Work out the finished part from the listing and answer in its coordinate system (mm). A direction names the side the tool comes from. Coordinates: 2 decimals unless noted, no trailing zeros. Loops run counter-clockwise (first coordinate to the right, second up) from the corner with the lowest first, then second, coordinate; pieces in that order, holes last. Notation, with made-up numbers: (-21, 0) -> (25, 0) arc R36 cw to (25, 39) -> close; hole circle Ø8 at (38.5, 82.5). An arc over 180 degrees is marked (long way). Use a Markdown table: item, result.
from build123d import *

# Parameters (mm, degrees)
SKETCH_1_R               = 2.5
EXTRUDE_1_DEPTH          = 25
CHAMFER_1_SIZE           = 0.5
CUT_EXTRUDE_1_DEPTH      = 26.248762346
CUT_EXTRUDE_1_DEPTH_BACK = 26.248762346
SKETCH_2_W               = 3.2
SKETCH_2_H               = 3.525136196


with BuildPart() as part:
    # 草图1 → 凸台-拉伸1 (new, symmetric)
    with BuildSketch(Plane.XY):
        Circle(SKETCH_1_R)
    extrude(amount=EXTRUDE_1_DEPTH, both=True)

    # 倒角1
    chamfer_1_edges = [part.edges().sort_by_distance(p)[0] for p in [
        (-2.5, 0, -25),
        (-2.5, 0, 25),
    ]]
    chamfer(chamfer_1_edges, length=CHAMFER_1_SIZE)

    # 草图2 → 切除-拉伸1 (cut, two sides: drawn at the far end of the back side and taken through both)
    with BuildSketch(Plane(origin=(0, 0, 0), x_dir=(0, 0, -1), z_dir=(1, 0, 0)).offset(-CUT_EXTRUDE_1_DEPTH_BACK)):
        with Locations((21.4, 3.262568098)):
            Rectangle(SKETCH_2_W, SKETCH_2_H)
    extrude(amount=CUT_EXTRUDE_1_DEPTH + CUT_EXTRUDE_1_DEPTH_BACK, mode=Mode.SUBTRACT)


solid = part.part
Q1. Given pin 1 Ø2 at (x, z) = (1.5, -9.5) entering from +Y, flat-ended and moving along its own axis, determine where the tip first touches the part or whether it passes through.
Solved:
| item | result |
|---|---|
| pin 1 | y = 2.45 |
Q2. Consider line 1 (Z direction, x = -0.2, y = 1.55); line 2 (Y direction, x = -1.4, z = -17.5); line 3 (X direction, y = 1.75, z = 1). Determine where each line is inside the solid, lowest interval first. Write a range as [from, to].
Solved:
| item | result |
|---|---|
| line 1 | [-25, -23], [-19.8, 25] |
| line 2 | [-2.07, 2.07] |
| line 3 | [-1.79, 1.79] |
Q3. Section A-A on z = 16 is taken. Determine the outline of the cut face in (x, y), and give its area (3 significant figures).
Solved:
| item | result |
|---|---|
| outline | circle Ø5 at (0, 0) |
| area | 19.6 mm² |
Q4. For faces 1 (the cylindrical face through (1.15, -2.22, 0.34)), 2 (the flat face through (0, 1.5, -21)), determine the directions among +Z, -Z, +X, -X, +Y, -Y from which every point of the face is accessible in a straight line to the end or side of a thin tool.
Solved:
| item | result |
|---|---|
| face 1 | +Z, -Z |
| face 2 | +X, -X, +Y |
Q5. Determine the mould class of faces 3 (the flat face through (0, 2, -19.8)), 4 (the flat face through (0, 0, 25)), 5 (the flat face through (0, 0, -25)) for opening direction Z: pulls with the +Z half, pulls with the -Z half, needs draft (parallel to the pull), parting line crosses it, or undercut.
Solved:
| item | result |
|---|---|
| face 3 | undercut |
| face 4 | pulls with the +Z half |
| face 5 | pulls with the -Z half |
